For this review, take the finished solid that the model builds, in its own axes (mm). A direction names the side the tool comes from. Coordinates: 2 decimals unless noted, no trailing zeros. Loops run counter-clockwise (first coordinate to the right, second up) from the corner with the lowest first, then second, coordinate; pieces in that order, holes last. Notation, with made-up numbers: (11.5, -25.5) -> (47.5, -25.5) arc R26 cw to (47.5, 11.5) -> close; hole circle Ø1 at (-21, -20). An arc over 180 degrees is marked (long way). Answer in a Markdown table with one row per item.
from build123d import *


with BuildPart() as part:
    # 草图1 → 旋转1 (revolve)
    with BuildSketch(Plane.XY, mode=Mode.PRIVATE) as revolve_1_sk:
        Polygon((7.5, 3), (7.5, 0), (9.5, 0), (9.5, -6), (10, -6), (10, -7), (9.5, -7), (9.5, -9), (20, -9), (20, -8), (16, -8), (16, 2), (20, 2), (20, 3), align=None)
    revolve(revolve_1_sk.sketch.rotate(Axis((0, 22.495377882, 0), (0, -1, 0)), 90), axis=Axis((0, 22.495377882, 0), (0, -1, 0)))


solid = part.part
Item 1: Take a section at C-C, the plane y = -3.5. State the section outline as (x, z) points.
Worked answers:
| item | result |
|---|---|
| outline | circle Ø32 at (0, 0); hole circle Ø19 at (0, 0) |
Item 2: Take a section at D-D, the plane x = 8.5. State the section outline as (y, z) points.
Worked answers:
| item | result |
|---|---|
| outline | (-9, -18.1) -> (-8, -18.1) -> (-8, -13.56) -> (2, -13.56) -> (2, -18.1) -> (3, -18.1) -> (3, 18.1) -> (2, 18.1) -> (2, 13.56) -> (-8, 13.56) -> (-8, 18.1) -> (-9, 18.1) -> (-9, 4.24) -> (-7, 4.24) -> (-7, 5.27) -> (-6, 5.27) -> (-6, 4.24) -> (0, 4.24) -> (0, -4.24) -> (-6, -4.24) -> (-6, -5.27) -> (-7, -5.27) -> (-7, -4.24) -> (-9, -4.24) -> close |
Item 3: For L1, parallel to X at y = 2.1, z = 0; L2, parallel to Y at x = 12, z = 15.5; L3, parallel to X at y = -6.5, z = 0, list the stretches that pass through material, from the lowest coordinate up.
Worked answers:
| item | result |
|---|---|
| L1 | -20 to -7.5, 7.5 to 20 |
| L2 | -9 to -8, 2 to 3 |
| L3 | -16 to -10, 10 to 16 |
Item 4: Take a section at B-B, the plane z = 0. State the section outline as (x, y) points, and give its area (3 significant figures).
Worked answers:
| item | result |
|---|---|
| outline | (-20, -9) -> (-9.5, -9) -> (-9.5, -7) -> (-10, -7) -> (-10, -6) -> (-9.5, -6) -> (-9.5, 0) -> (-7.5, 0) -> (-7.5, 3) -> (-20, 3) -> (-20, 2) -> (-16, 2) -> (-16, -8) -> (-20, -8) -> close; (7.5, 0) -> (9.5, 0) -> (9.5, -6) -> (10, -6) -> (10, -7) -> (9.5, -7) -> (9.5, -9) -> (20, -9) -> (20, -8) -> (16, -8) -> (16, 2) -> (20, 2) -> (20, 3) -> (7.5, 3) -> close |
| area | 183 mm² |
Item 5: Insertion check: pin 1 (4 mm diameter, centred on x = 14.5, y = -7.5, fed in from +Z); pin 2 (10 mm diameter, centred on x = 2, z = -0.5, fed in from -Y); pin 3 (5 mm diameter, centred on x = 7.5, y = 1, fed in from +Z); pin 4 (3 mm diameter, centred on x = 12.5, y = 0, fed in from +Z). Each pin has a flat end and moves straight along its axis. Give the tip position at first contact, or say it passes through.
Worked answers:
| item | result |
|---|---|
| pin 1 | z = 15.56 |
| pin 2 | through |
| pin 3 | z = 19.31 |
| pin 4 | z = 11.62 |
Item 6: Take a section at A-A, the plane x = 0. State the section outline as (y, z) points, and give its area (3 significant figures).
Worked answers:
| item | result |
|---|---|
| outline | (-9, -20) -> (-8, -20) -> (-8, -16) -> (2, -16) -> (2, -20) -> (3, -20) -> (3, -7.5) -> (0, -7.5) -> (0, -9.5) -> (-6, -9.5) -> (-6, -10) -> (-7, -10) -> (-7, -9.5) -> (-9, -9.5) -> close; (-9, 9.5) -> (-7, 9.5) -> (-7, 10) -> (-6, 10) -> (-6, 9.5) -> (0, 9.5) -> (0, 7.5) -> (3, 7.5) -> (3, 20) -> (2, 20) -> (2, 16) -> (-8, 16) -> (-8, 20) -> (-9, 20) -> close |
| area | 183 mm² |
Item 7: For faces 4 (the cylindrical face through (9.274, -8.014, -2.059)), 5 (the cylindrical face through (-0.88, 2.51, -19.98)), 6 (the flat face through (4, -6, -9)), list the 3-axis set-ups (+Z, -Z, +X, -X, +Y, -Y) from which the entire face can be reached by the end or side of a thin tool; tool diameter is ignored.
Worked answers:
| item | result |
|---|---|
| face 4 | -Y |
| face 5 | +Y, -Y |
| face 6 | none |
Item 8: The part is to be moulded in two halves that separate along X. For faces 1 (the cylindrical face through (15.62, -2.93, -3.47)), 2 (the flat face through (0, 3, 9)), 3 (the flat face through (-8, 0, -1)), say which applies: +X half, -X half, draft (parallel to the pull), parting line (faces both ways), or undercut.
Worked answers:
| item | result |
|---|---|
| face 1 | parting line |
| face 2 | draft |
| face 3 | undercut |
